Answer from the drawing. Dimensions are ordinates in mm from the lowest x, y and z of the part. A direction names the side the tool comes from. Give positions to 0.01 mm unless a question says otherwise; leave off trailing zeros. Write each loop counter-clockwise with the first axis right and the second up, starting at its lowest first coordinate (ties: lowest second). Pieces come first, ordered by that corner, then holes. Notation, with made-up numbers: M 7,62.25 L 32,62.25 A21 ccw 32,95.25 Z; hole C 82.25,60 d11. An arc over 180 degrees is marked long. Put each result on its own line as item: value.
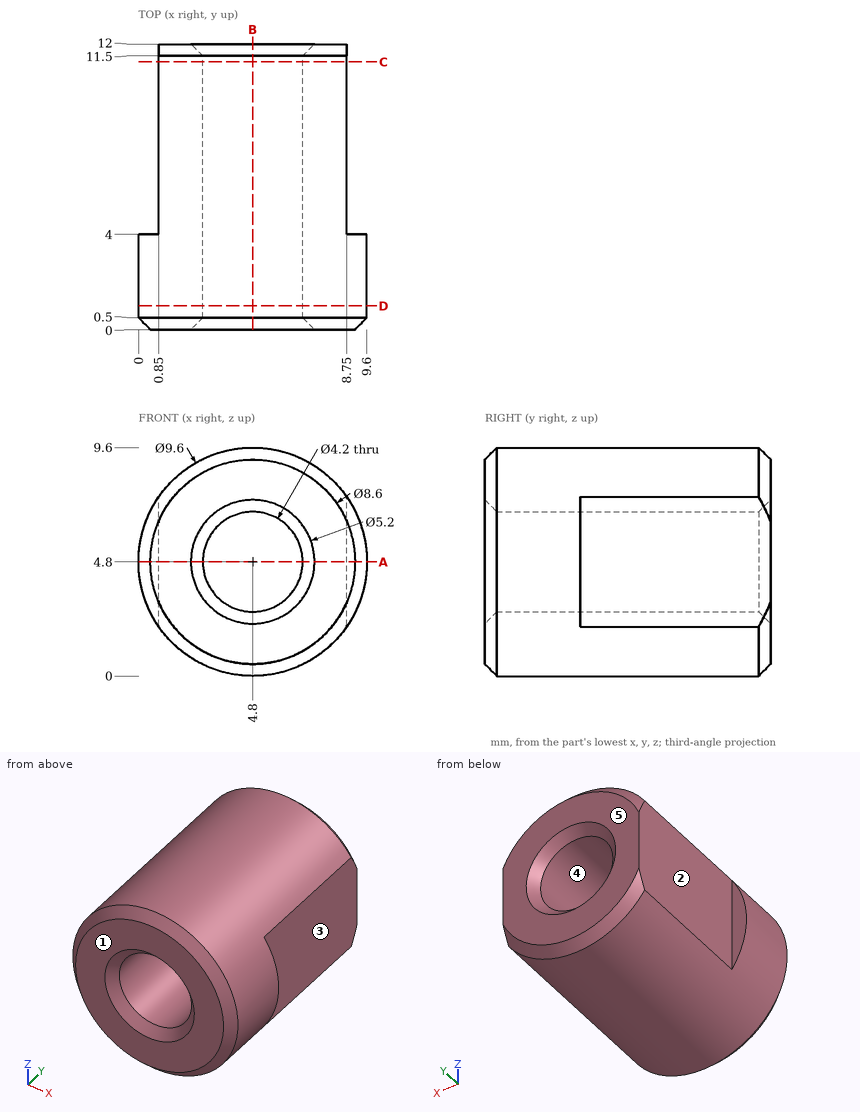
(1) Section C-C on y = 11.25 is taken. Determine the outline of the cut face in (x, z).
Result:
outline: M 0.85,2.07 A4.8 ccw 8.75,2.07 L 8.75,7.53 A4.8 ccw 0.85,7.53 Z; hole C 4.8,4.8 d4.2
(2) Given pin 1 Ø1.5 at (x, y) = (7, 4) entering from +Z; pin 2 Ø4.5 at (y, z) = (6.5, 5.5) entering from +X; pin 3 Ø2.5 at (x, z) = (4.8, 4.8) entering from +Y; pin 4 Ø2.5 at (y, z) = (8, 4.5) entering from -X, each flat-ended and moving along its own axis, determine where each tip first touches the part or whether it passes through.
Result:
pin 1: stops at z = 9.38
pin 2: stops at x = 8.75
pin 3: passes through
pin 4: stops at x = 0.85
(3) Straight lines are drawn through the part: line 1 along X through (y, z) = (9.5, 4.8); line 2 along X through (y, z) = (3.5, 4.8); line 3 along Z through (x, y) = (4.5, 9.5). For each, find the intervals that lie inside material, in ascending order. Write a range as from..to.
Result:
line 1: x = 0.85..2.7, 6.9..8.75
line 2: x = 0..2.7, 6.9..9.6
line 3: z = 0.01..2.72, 6.88..9.59
(4) Section D-D on y = 1 is taken. Determine the outline of the cut face in (x, z), and give its area (3 significant figures).
Result:
outline: C 4.8,4.8 d9.6; hole C 4.8,4.8 d4.2
area: 58.5 mm²
(5) Section A-A on z = 4.8 is taken. Determine the outline of the cut face in (x, y).
Result:
outline: M 0,0.5 L 0.5,0 L 2.2,0 L 2.7,0.5 L 2.7,11.5 L 2.2,12 L 0.85,12 L 0.85,4 L 0,4 Z; M 6.9,0.5 L 7.4,0 L 9.1,0 L 9.6,0.5 L 9.6,4 L 8.75,4 L 8.75,12 L 7.4,12 L 6.9,11.5 Z
(6) For a pull along X with two mould halves and no side action, classify the marked faces 3, 4 and 5 as +X half, -X half, draft (parallel to the pull), parting line (faces both ways), or undercut.
Result:
face 3: +X half
face 4: undercut
face 5: draft
(7) Which of the six approach directions +Z, -Z, +X, -X, +Y, -Y give full straight-line access (tool end or side, diameter ignored) to the marked faces 1 and 2?
Result:
face 1: +Z, -Z, +X, -X, -Y
face 2: +Z, -Z, -X, +Y
(8) Section B-B on x = 4.8 is taken. Determine the outline of the cut face in (y, z), and give its area (3 significant figures).
Result:
outline: M 0,0.5 L 0.5,0 L 11.5,0 L 12,0.5 L 12,2.2 L 11.5,2.7 L 0.5,2.7 L 0,2.2 Z; M 0,7.4 L 0.5,6.9 L 11.5,6.9 L 12,7.4 L 12,9.1 L 11.5,9.6 L 0.5,9.6 L 0,9.1 Z
area: 63.8 mm²
